from build123d import *

# Parameters (mm, degrees)
SKETCH1_R           = 10
BOSS_EXTRUDE1_DEPTH = 2.5
SKETCH5_R           = 1
SKETCH7_R           = 1


with BuildPart() as part:
    # Sketch1 → Boss-Extrude1 (new, symmetric)
    with BuildSketch(Plane.XY):
        Circle(SKETCH1_R)
    extrude(amount=BOSS_EXTRUDE1_DEPTH, both=True)

    # Sweep1: sweep along a path in Sketch3
    with BuildLine(Plane(origin=(0, 0, 0), x_dir=(1, 0, 0), z_dir=(0, 1, 0))) as sweep1_path:
        Line((-4.078135837, 6.578135837), (0, 2.5))
        Line((0, 2.5), (3.535533906, 6.035533906))
    # Sketch5 → Sweep1 (sweep)
    with BuildSketch(Plane(origin=(3.535533906, 0, -6.035533906), x_dir=(-0.7071067811865517, 0, -0.7071067811865434), z_dir=(0.7071067811865434, 0, -0.7071067811865517))):
        Circle(SKETCH5_R)
    sweep(path=sweep1_path.line, transition=Transition.RIGHT)

    # Sweep2: sweep along a path in Sketch8
    with BuildLine(Plane(origin=(0, 0, 0), x_dir=(1, 0, 0), z_dir=(0, 1, 0))) as sweep2_path:
        Line((3.535533906, 6.035533906), (0, 2.5))
        Line((0, 2.5), (-2.595836944, -2.5))
        Line((-2.595836944, -2.5), (-6.619258355, -6.523421411))
    # Sketch7 → Sweep2 (sweep)
    with BuildSketch(Plane(origin=(-6.619258355, 0, 6.523421411), x_dir=(0.7071067811865527, 0, 0.7071067811865425), z_dir=(-0.7071067811865425, 0, 0.7071067811865527))):
        Circle(SKETCH7_R)
    sweep2 = sweep(path=sweep2_path.line, transition=Transition.RIGHT)

    # Mirror1: Sweep2 across plane
    add(sweep2.mirror(Plane(origin=(0, 0, 0), x_dir=(0, 0, 1), z_dir=(1, 0, 0))))


solid = part.part
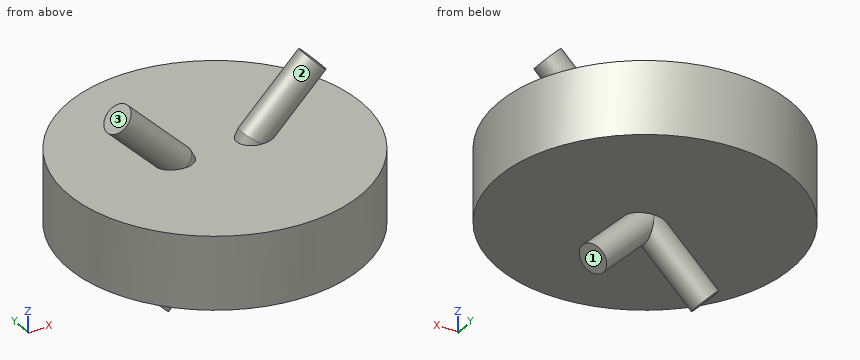
Can you work these out from the model? Positions are in its coordinate system, mm. Face numbers are marked on the shaded views. Coordinates: 2 decimals unless noted, no trailing zeros. Loops run counter-clockwise (first coordinate to the right, second up) from the corner with the lowest first, then second, coordinate; pieces in that order, holes last. Notation, with made-up numbers: (-2, 27) - (2, 27) arc R25 cw to (2, 41) - close; hole circle Ø1 at (46.25, -26.5). An arc over 180 degrees is marked (long way). Put each result on its own line as item: value. Start each with the question number.
Item 1: Suppose I cut it at B-B (y = 9.25). Please give me the cut outline in (x, z).
Item 2: If we mould it in two halves opening along Z, with no side actions, what happens to the marked faces 1, 2 and 3? For each: +Z half, -Z half, draft (parallel to the pull), parting line (faces both ways), or undercut.
Item 3: If I drill on line 1 along Z through (x, y) = (2.75, 1.5); line 2 along Y through (x, z) = (-6.5, -1.75); line 3 along X through (y, z) = (3.25, -1.75), over which ranges is the centre line in solid material (lowest first)?
Item 4: Suppose I cut it at C-C (y = 5.75). Please give me the cut outline in (x, z), and give its area (3 significant figures).
Item 5: For pin 1 (6 mm diameter, centred on x = 3.5, y = 2.5, fed in from +Z); pin 2 (6 mm diameter, centred on x = -5.5, z = -2.5, fed in from +Y); pin 3 (10 mm diameter, centred on x = 1.5, y = -3, fed in from -Z), each with a flat end and sliding along its axis, tell me the tip position at first contact or that it passes through.
Item 6: Suppose I cut it at A-A (y = 0). Please give me the cut outline in (x, z), and give its area (3 significant figures).
Here are the results:
1. outline: (-3.8, -2.5) - (3.8, -2.5) - (3.8, 2.5) - (-3.8, 2.5) - close
2. face 1: -Z half
2. face 2: undercut
2. face 3: +Z half
3. line 1: -2.5 to 2.5
3. line 2: -7.6 to 7.6
3. line 3: -9.46 to 9.46
4. outline: (-8.18, -2.5) - (8.18, -2.5) - (8.18, 2.5) - (-8.18, 2.5) - close
4. area: 81.8 mm²
5. pin 1: z = 6.87
5. pin 2: y = 9.68
5. pin 3: z = -6.74
6. outline: (-10, -2.5) - (-1.41, -2.5) - (-4.79, -5.87) - (-3.37, -7.29) - (0, -3.91) - (2.83, -6.74) - (4.24, -5.33) - (1.41, -2.5) - (10, -2.5) - (10, 2.5) - (4.01, 2.5) - (7.33, 5.82) - (5.91, 7.23) - (1.78, 3.1) - (1.47, 2.5) - (-1.47, 2.5) - (-1.78, 3.1) - (-5.91, 7.23) - (-7.33, 5.82) - (-4.01, 2.5) - (-10, 2.5) - close
6. area: 142 mm²
